Answer from the drawing. Dimensions are ordinates in mm from the lowest x, y and z of the part. A direction names the side the tool comes from. Round coordinates to 2 decimals unless told otherwise and drop trailing zeros. Order: outer loops, then holes, each group sorted by start corner. A loop starts at its lowest first (then second) coordinate and runs counter-clockwise, first axis right, second up.
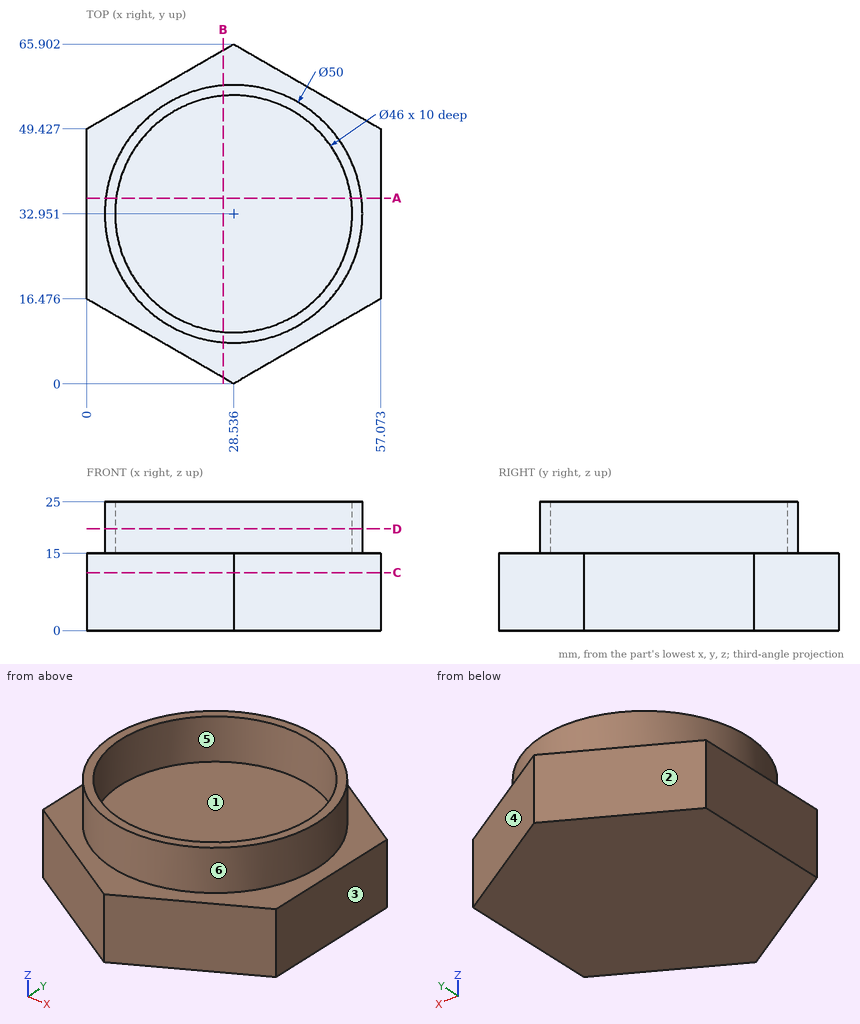
Q1. A cutting plane is placed at D-D, the plane z = 19.75. Give the vertices of the cut face in (x, y).
Outcome:
outline: circle Ø50 at (28.54, 32.95); hole circle Ø46 at (28.54, 32.95)
Q2. A cutting plane is placed at A-A, the plane y = 36. Give the vertices of the cut face in (x, z).
Outcome:
outline: (0, 0) - (57.07, 0) - (57.07, 15) - (53.35, 15) - (53.35, 25) - (51.33, 25) - (51.33, 15) - (5.74, 15) - (5.74, 25) - (3.72, 25) - (3.72, 15) - (0, 15) - close
Q3. Flat-ended cylindrical pins translate along their axes: pin 1 (8 mm diameter, centred on x = 9.5, y = 48, fed in from -Z); pin 2 (4 mm diameter, centred on x = 20.5, z = 5.5, fed in from +Y); pin 3 (17 mm diameter, centred on x = 23.5, y = 20.5, fed in from +Z); pin 4 (1 mm diameter, centred on x = 49, z = 17, fed in from -Y) (1 decimal). Find the tip coordinate at first contact, or state that the pin passes through.
Outcome:
pin 1: stops at z = 0
pin 2: stops at y = 62.42
pin 3: stops at z = 15
pin 4: stops at y = 17.9
Q4. A cutting plane is placed at C-C, the plane z = 11.25. Give the vertices of the cut face in (x, y) (1 decimal).
Outcome:
outline: (0, 16.5) - (28.5, 0) - (57.1, 16.5) - (57.1, 49.4) - (28.5, 65.9) - (0, 49.4) - close
Q5. For the marked faces 1 and 2, determine the directions among +Z, -Z, +X, -X, +Y, -Y from which every point of the face is accessible in a straight line to the end or side of a thin tool.
Outcome:
face 1: +Z
face 2: +Z, -Z, -X, +Y
Q6. Straight lines are drawn through the part: probe 1 along Z at (x, y) = (14, 54.5); probe 2 along Y at (x, z) = (35, 24) (1 decimal); probe 3 along Y at (x, z) = (47.5, 21.5) (1 decimal). For each, find the intervals that lie inside material, in ascending order.
Outcome:
probe 1: z = 0 to 15
probe 2: y = 8.8 to 10.9, 55 to 57.1
probe 3: y = 16.7 to 19.9, 46 to 49.2
Q7. For a pull along Y with two mould halves and no side action, classify the marked faces 3, 4, 5 and 6 as released by +Y, released by -Y, zero draft, split by the parting line, or undercut.
Outcome:
face 3: zero draft
face 4: released by +Y
face 5: undercut
face 6: split by the parting line
Q8. A cutting plane is placed at B-B, the plane x = 26.5. Give the vertices of the cut face in (y, z) (1 decimal).
Outcome:
outline: (1.2, 0) - (64.7, 0) - (64.7, 15) - (57.9, 15) - (57.9, 25) - (55.9, 25) - (55.9, 15) - (10, 15) - (10, 25) - (8, 25) - (8, 15) - (1.2, 15) - close
